For this review, use the dimensioned drawing (mm, ordinates from the lowest corner) and the shaded views. A direction names the side the tool comes from. Give positions to 0.01 mm unless a question says otherwise; leave off trailing zeros. Order: outer loops, then holes, each group sorted by start corner. A loop starts at its lowest first (then second) coordinate and runs counter-clockwise, first axis right, second up.
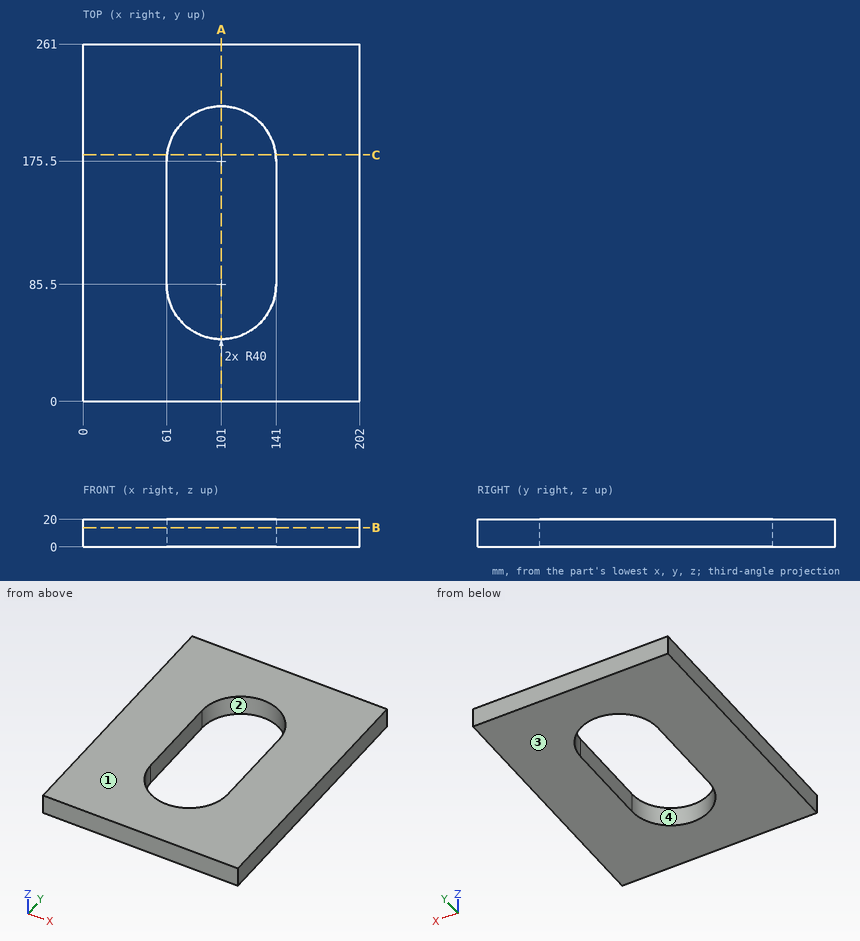
1. Draft analysis for pull direction Y (two halves, no side actions). For the marked faces 1 and 2, state which applies: pulls with the +Y half, pulls with the -Y half, needs draft (parallel to the pull), parting line crosses it, or undercut.
2. Take a section at C-C (y = 180). Write out the cut boundary in (x, z), and give its area (3 significant figures).
3. For the marked faces 3 and 4, list the 3-axis set-ups (+Z, -Z, +X, -X, +Y, -Y) from which the entire face can be reached by the end or side of a thin tool; tool diameter is ignored.
4. To check wall thickness, follow line 1 (Y direction, x = 75, z = 7); line 2 (X direction, y = 105.5, z = 17.5); line 3 (Y direction, x = 102, z = 6.5). State the ranges of each line that lie inside material, in increasing order.
5. Take a section at B-B (z = 14). Write out the cut boundary in (x, y).
6. Take a section at A-A (x = 101). Write out the cut boundary in (y, z), and give its area (3 significant figures).
Answer:
1. face 1: needs draft
1. face 2: undercut
2. outline: (0, 0) - (61.25, 0) - (61.25, 20) - (0, 20) - close; (140.75, 0) - (202, 0) - (202, 20) - (140.75, 20) - close
2. area: 2,450 mm2
3. face 3: -Z, +X, -X, +Y, -Y
3. face 4: +Z, -Z
4. line 1: y = 0 to 55.1, 205.9 to 261
4. line 2: x = 0 to 61, 141 to 202
4. line 3: y = 0 to 45.51, 215.49 to 261
5. outline: (0, 0) - (202, 0) - (202, 261) - (0, 261) - close; hole (61, 85.5) arc R40 ccw to (141, 85.5) - (141, 175.5) arc R40 ccw to (61, 175.5) - close
6. outline: (0, 0) - (45.5, 0) - (45.5, 20) - (0, 20) - close; (215.5, 0) - (261, 0) - (261, 20) - (215.5, 20) - close
6. area: 1,820 mm2
